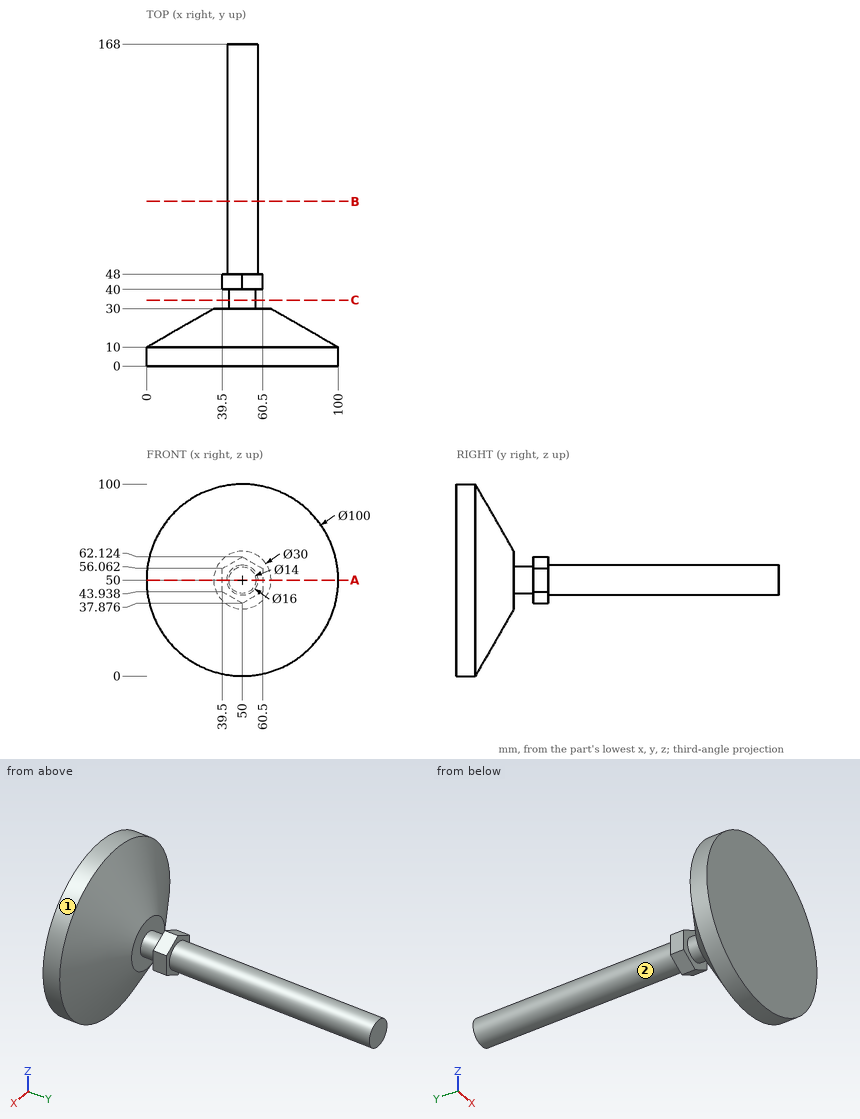
Check sheet for the drawn part. Datum: minimum x, y, z corner. Units: mm. A direction names the side the tool comes from. Give positions to 0.01 mm unless a question says otherwise; leave off trailing zeros. Order: outer loops, then holes, each group sorted by start corner. A loop starts at its lowest first (then second) coordinate and runs counter-clockwise, first axis right, second up. Notation, with made-up numbers: (60.25, -34) - (86.25, -34) arc R25 cw to (86.25, -22) - close; hole circle Ø9 at (27.5, 21.25). An arc over 180 degrees is marked (long way). Answer in a Markdown table with one row per item. Add a question column.
Q1. Material ranges on probe 1 along X at (y, z) = (8.5, 73.5); probe 2 along X at (y, z) = (131.5, 46.5) (1 decimal); probe 3 along Z at (x, y) = (52.5, 141.5), recorded low to high. Write a range as from..to.
Q2. Tool access check on the marked faces 1 and 2. Record the directions out of +Z, -Z, +X, -X, +Y, -Y that give a thin tool (end or side, any length) a straight path to the whole face; none if there is none.
Q3. Cross-section at A-A, the plane z = 50. Enter the section's corners in (x, y), then the cut area to 3 significant figures.
Q4. Cross-section at B-B, the plane y = 86. Enter the section's corners in (x, z).
Q5. Gauge pin test, flat ends, axial feed: pin 1 (2.5 mm diameter, centred on y = 44.5, z = 51, fed in from +X); pin 2 (5 mm diameter, centred on x = 51, y = 39, fed in from -Z); pin 3 (3 mm diameter, centred on y = 46, z = 62.5, fed in from -X). Record the tip position at first contact, or that the pin passes through.
Q6. Cross-section at C-C, the plane y = 34.5. Enter the section's corners in (x, z), then the cut area to 3 significant figures.
Check values:
| question | item | result |
|---|---|---|
| 1 | probe 1 | x = 5.87..94.13 |
| 1 | probe 2 | x = 42.8..57.2 |
| 1 | probe 3 | z = 42.4..57.6 |
| 2 | face 1 | +Y, -Y |
| 2 | face 2 | +Y |
| 3 | outline | (0, 0) - (100, 0) - (100, 10) - (65, 30) - (57, 30) - (57, 40) - (60.5, 40) - (60.5, 48) - (58, 48) - (58, 168) - (42, 168) - (42, 48) - (39.5, 48) - (39.5, 40) - (43, 40) - (43, 30) - (35, 30) - (0, 10) - close |
| 3 | area | 4,530 mm^2 |
| 4 | outline | circle Ø16 at (50, 50) |
| 5 | pin 1 | stops at x = 60.5 |
| 5 | pin 2 | stops at z = 37.88 |
| 5 | pin 3 | stops at x = 48.05 |
| 6 | outline | circle Ø14 at (50, 50) |
| 6 | area | 154 mm^2 |
